For this review, take the finished solid that the model builds, in its own axes (mm). A direction names the side the tool comes from. Coordinates: 2 decimals unless noted, no trailing zeros. Loops run counter-clockwise (first coordinate to the right, second up) from the corner with the lowest first, then second, coordinate; pieces in that order, holes last. Notation, with made-up numbers: M 31.25,44 L 36.25,44 A33 ccw 36.25,81 Z; hole C 67.5,14.5 d5. An arc over 180 degrees is marked long. Write item = value, one per line.
from build123d import *

# Parameters (mm, degrees)
SKETCH1_W           = 2.9
SKETCH1_H           = 20
BOSS_EXTRUDE1_DEPTH = 3
FILLET1_R           = 5
FILLET2_R           = 30
CUT_EXTRUDE1_REACH  = 166.165
SKETCH3_R           = 7.5
SKETCH3_R_2         = 2.3
SKETCH5_W           = 20
SKETCH5_H           = 2.9
CUT_EXTRUDE2_DEPTH  = 3
SKETCH6_R           = 2.3
CUT_EXTRUDE3_DEPTH  = 3


with BuildPart() as part:
    # Sketch1 → Boss-Extrude1 (new body)
    with BuildSketch(Plane.XY):
        Polygon((0, 0), (-23, 0), (-23, 68), (-75, 143), (-47.5, 143), (-47.5, 146), (-27.5, 146), (-27.5, 143), (0, 143), align=None)
        with Locations((-16.5, 15)):
            Rectangle(SKETCH1_W, SKETCH1_H, mode=Mode.SUBTRACT)
        with Locations((-6.5, 15)):
            Rectangle(SKETCH1_W, SKETCH1_H, mode=Mode.SUBTRACT)
    extrude(amount=BOSS_EXTRUDE1_DEPTH)

    # Fillet1
    fillet1_edges = [part.edges().sort_by_distance(p)[0] for p in [
        (0, 0, 1.5),
        (-23, 0, 1.5),
    ]]
    fillet(fillet1_edges, radius=FILLET1_R)

    # Fillet2
    fillet2_edges = [part.edges().sort_by_distance(p)[0] for p in [
        (-23, 68, 1.5),
    ]]
    fillet(fillet2_edges, radius=FILLET2_R)

    # Sketch3 → Cut-Extrude1 (cut, up to next)
    with BuildSketch(Plane(origin=(0, 0, 0), x_dir=(-1, 0, 0), z_dir=(0, 0, -1)), mode=Mode.PRIVATE) as cut_extrude1_sk1:
        with Locations((12, 73)):
            Circle(SKETCH3_R)
    cut_extrude1_tool1 = extrude(cut_extrude1_sk1.sketch, amount=-CUT_EXTRUDE1_REACH, mode=Mode.PRIVATE) & part.part
    # Sketch3 → Cut-Extrude1 (cut, up to next)
    with BuildSketch(Plane(origin=(0, 0, 0), x_dir=(-1, 0, 0), z_dir=(0, 0, -1)), mode=Mode.PRIVATE) as cut_extrude1_sk2:
        with Locations((17.05, 59.5)):
            Circle(SKETCH3_R_2)
    cut_extrude1_tool2 = extrude(cut_extrude1_sk2.sketch, amount=-CUT_EXTRUDE1_REACH, mode=Mode.PRIVATE) & part.part
    # Sketch3 → Cut-Extrude1 (cut, up to next)
    with BuildSketch(Plane(origin=(0, 0, 0), x_dir=(-1, 0, 0), z_dir=(0, 0, -1)), mode=Mode.PRIVATE) as cut_extrude1_sk3:
        with Locations((6.95, 59.5)):
            Circle(SKETCH3_R_2)
    cut_extrude1_tool3 = extrude(cut_extrude1_sk3.sketch, amount=-CUT_EXTRUDE1_REACH, mode=Mode.PRIVATE) & part.part
    # Sketch3 → Cut-Extrude1 (cut, up to next)
    with BuildSketch(Plane(origin=(0, 0, 0), x_dir=(-1, 0, 0), z_dir=(0, 0, -1)), mode=Mode.PRIVATE) as cut_extrude1_sk4:
        with Locations((17.05, 109.5)):
            Circle(SKETCH3_R_2)
    cut_extrude1_tool4 = extrude(cut_extrude1_sk4.sketch, amount=-CUT_EXTRUDE1_REACH, mode=Mode.PRIVATE) & part.part
    # Sketch3 → Cut-Extrude1 (cut, up to next)
    with BuildSketch(Plane(origin=(0, 0, 0), x_dir=(-1, 0, 0), z_dir=(0, 0, -1)), mode=Mode.PRIVATE) as cut_extrude1_sk5:
        with Locations((6.95, 109.5)):
            Circle(SKETCH3_R_2)
    cut_extrude1_tool5 = extrude(cut_extrude1_sk5.sketch, amount=-CUT_EXTRUDE1_REACH, mode=Mode.PRIVATE) & part.part
    add(cut_extrude1_tool1.solids().sort_by_distance((-12, 73, 0))[0], mode=Mode.SUBTRACT)
    add(cut_extrude1_tool2.solids().sort_by_distance((-17.05, 59.5, 0))[0], mode=Mode.SUBTRACT)
    add(cut_extrude1_tool3.solids().sort_by_distance((-6.95, 59.5, 0))[0], mode=Mode.SUBTRACT)
    add(cut_extrude1_tool4.solids().sort_by_distance((-17.05, 109.5, 0))[0], mode=Mode.SUBTRACT)
    add(cut_extrude1_tool5.solids().sort_by_distance((-6.95, 109.5, 0))[0], mode=Mode.SUBTRACT)

    # Sketch5 → Cut-Extrude2 (cut)
    with BuildSketch(Plane(origin=(0, 0, 0), x_dir=(-1, 0, 0), z_dir=(0, 0, -1))):
        with Locations((15, 98)):
            Rectangle(SKETCH5_W, SKETCH5_H)
    extrude(amount=-CUT_EXTRUDE2_DEPTH, mode=Mode.SUBTRACT)

    # Sketch6 → Cut-Extrude3 (cut)
    with BuildSketch(Plane.XY.offset(3)):
        with Locations((-17.05, 39.5)):
            Circle(SKETCH6_R)
        with Locations((-6.95, 39.5)):
            Circle(SKETCH6_R)
    extrude(amount=-CUT_EXTRUDE3_DEPTH, mode=Mode.SUBTRACT)


solid = part.part
Q1. For line 1 along X through (y, z) = (7, 2); line 2 along Y through (x, z) = (-15, 1.25); line 3 along Y through (x, z) = (-13.5, 1.1), list the stretches that pass through material, from the lowest coordinate up.
Solved:
line_1 = -23 to -17.95, -15.05 to -7.95, -5.05 to 0
line_2 = 0 to 38.46, 40.54 to 58.46, 60.54 to 66.13, 79.87 to 96.55, 99.45 to 108.46, 110.54 to 143
line_3 = 0 to 65.65, 80.35 to 96.55, 99.45 to 143
Q2. Machinability: for faces 1 (the face through (-24.33, 67.45, 1.52)), 2 (the face through (-15, 99.45, 1)), 3 (the face through (-20, 90, 3)), 4 (the face through (-14, 143, 1)), 5 (the face through (-61, 143, 1)), which of the approach directions +Z, -Z, +X, -X, +Y, -Y give a long, thin tool a straight path to every point of the face, cutting with its end or side? Answer none if there is none.
Solved:
face_1 = +Z, -Z, -X, -Y
face_2 = +Z, -Z
face_3 = +Z, +X, -X, +Y, -Y
face_4 = +Z, -Z, +X, +Y
face_5 = +Z, -Z, -X, +Y
Q3. For pin 1 Ø1 at (x, z) = (-38.5, 2.5) entering from -Y; pin 2 Ø1.5 at (x, z) = (-55.5, 1) entering from +Y; pin 3 Ø1 at (x, z) = (-22.5, 2) entering from -Y, all flat-tipped, find the tip position at first contact; note any pin that passes through.
Solved:
pin_1 = 89.63
pin_2 = 143
pin_3 = 2
Q4. Add section B-B (y = 39.5). Write out the cut boundary in (x, z), and give its area (3 significant figures).
Solved:
outline = M -23,0 L -19.35,0 L -19.35,3 L -23,3 Z; M -14.75,0 L -9.25,0 L -9.25,3 L -14.75,3 Z; M -4.65,0 L 0,0 L 0,3 L -4.65,3 Z
area = 41.4 mm²
Q5. Draft analysis for pull direction X (two halves, no side actions). For faces 6 (the face through (-21, 1, 2)), 7 (the face through (-17, 5, 1)), 8 (the face through (-15, 96.55, 1)), 9 (the face through (-20, 90, 0)), state which applies: +X half, -X half, draft (parallel to the pull), parting line (faces both ways), or undercut.
Solved:
face_6 = -X half
face_7 = undercut
face_8 = undercut
face_9 = draft
Q6. Add section D-D (y = 73). Write out the cut boundary in (x, z), and give its area (3 significant figures).
Solved:
outline = M -26.67,0 L -19.5,0 L -19.5,3 L -26.67,3 Z; M -4.5,0 L 0,0 L 0,3 L -4.5,3 Z
area = 35.0 mm²
Q7. Add section A-A (x = -12). Write out the cut boundary in (y, z).
Solved:
outline = M 0,0 L 65.5,0 L 65.5,3 L 0,3 Z; M 80.5,0 L 96.55,0 L 96.55,3 L 80.5,3 Z; M 99.45,0 L 143,0 L 143,3 L 99.45,3 Z
Q8. Add section C-C (z = 0.8). State how many separate pieces and enclosed holes the cut face has, and give its area (3 significant figures).
Solved:
separate_pieces = 1
enclosed_holes = 10
area = 4,850 mm²
